Can you work these out from the model? Positions are in its coordinate system, mm. Round coordinates to 2 decimals unless told otherwise and drop trailing zeros. Use a Markdown table: item, result. Add a question column.
```python
from build123d import *

# Parameters (mm, degrees)
SKETCH_1_R      = 2.1
SKETCH_1_R_2    = 3.4
EXTRUDE_1_DEPTH = 1940


with BuildPart() as part:
    # 草图1 → 拉伸1 (new body)
    with BuildSketch(Plane(origin=(0, 0, 0), x_dir=(1, 0, 0), z_dir=(0, 1, 0))):
        with BuildLine():
            Line((6.75, -28), (11, -28))
            Line((11, -28), (11, -30))
            Line((11, -30), (2, -30))
            ThreePointArc((2, -30), (0.585786438, -29.414213562), (0, -28))
            Line((0, -28), (0, -19))
            Line((0, -19), (2, -19))
            Line((2, -19), (2, -23.25))
            Line((2, -23.25), (5.335785999, -23.25))
            Line((5.335785999, -23.25), (9, -19.585785999))
            Line((9, -19.585785999), (9, -10.414214001))
            Line((9, -10.414214001), (5.335785999, -6.75))
            Line((5.335785999, -6.75), (2, -6.75))
            Line((2, -6.75), (2, -11))
            Line((2, -11), (0, -11))
            Line((0, -11), (0, -2))
            ThreePointArc((0, -2), (0.585786438, -0.585786438), (2, 0))
            Line((2, 0), (11, 0))
            Line((11, 0), (11, -2))
            Line((11, -2), (6.75, -2))
            Line((6.75, -2), (6.75, -5.335785999))
            Line((6.75, -5.335785999), (10.414214001, -9))
            Line((10.414214001, -9), (19.585785999, -9))
            Line((19.585785999, -9), (23.25, -5.335785999))
            Line((23.25, -5.335785999), (23.25, -2))
            Line((23.25, -2), (19, -2))
            Line((19, -2), (19, 0))
            Line((19, 0), (28, 0))
            ThreePointArc((28, 0), (29.414213562, -0.585786438), (30, -2))
            Line((30, -2), (30, -11))
            Line((30, -11), (28, -11))
            Line((28, -11), (28, -6.75))
            Line((28, -6.75), (24.664214001, -6.75))
            Line((24.664214001, -6.75), (21, -10.414214001))
            Line((21, -10.414214001), (21, -19.585785999))
            Line((21, -19.585785999), (24.664214001, -23.25))
            Line((24.664214001, -23.25), (28, -23.25))
            Line((28, -23.25), (28, -19))
            Line((28, -19), (30, -19))
            Line((30, -19), (30, -28))
            ThreePointArc((30, -28), (29.414213562, -29.414213562), (28, -30))
            Line((28, -30), (19, -30))
            Line((19, -30), (19, -28))
            Line((19, -28), (23.25, -28))
            Line((23.25, -28), (23.25, -24.664214001))
            Line((23.25, -24.664214001), (19.585785999, -21))
            Line((19.585785999, -21), (10.414214001, -21))
            Line((10.414214001, -21), (6.75, -24.664214001))
            Line((6.75, -24.664214001), (6.75, -28))
        make_face()
        with Locations(Location((3.375, -26.625, 0), (0, 0, 270))):
            Circle(SKETCH_1_R, mode=Mode.SUBTRACT)
        with Locations(Location((26.625, -26.625, 0), (0, 0, 270))):
            Circle(SKETCH_1_R, mode=Mode.SUBTRACT)
        with Locations(Location((15, -15, 0), (0, 0, 270))):
            Circle(SKETCH_1_R_2, mode=Mode.SUBTRACT)
        with Locations(Location((3.375, -3.375, 0), (0, 0, 270))):
            Circle(SKETCH_1_R, mode=Mode.SUBTRACT)
        with Locations(Location((26.625, -3.375, 0), (0, 0, 270))):
            Circle(SKETCH_1_R, mode=Mode.SUBTRACT)
    extrude(amount=EXTRUDE_1_DEPTH)


solid = part.part
```
(1) Suppose I cut it at A-A on y = 1342. Count the separate pieces of the cut face and the enclosed holes in it, and give its area (3 significant figures).
(2) I'm going to push flat-ended pins straight in: pin 1 (1 mm diameter, centred on x = 1, y = 498.5, fed in from +Z); pin 2 (1.6 mm diameter, centred on y = 528.5, z = 29, fed in from +X); pin 3 (5.5 mm diameter, centred on x = 15, z = 15, fed in from +Y); pin 4 (7.5 mm diameter, centred on x = 15, y = 671, fed in from +Z). Where does each tip first touch, or does it pass through?
(3) If I drill on probe 1 along X at (y, z) = (1275, 25.25); probe 2 along Z at (x, y) = (7.25, 810); probe 3 along Z at (x, y) = (3.5, 1173.5), over which ranges is the centre line in solid material (lowest first)? Write a range as [from, to].
Results below:
| question | item | result |
|---|---|---|
| 1 | separate pieces | 1 |
| 1 | enclosed holes | 5 |
| 1 | area | 333 mm² |
| 2 | pin 1 | stops at z = 29.94 |
| 2 | pin 2 | stops at x = 29.99 |
| 2 | pin 3 | passes through |
| 2 | pin 4 | stops at z = 21 |
| 3 | probe 1 | x = [0, 1.79], [4.96, 6.75], [23.25, 25.04], [28.21, 30] |
| 3 | probe 2 | z = [0, 2], [5.84, 8.66], [21.34, 24.16], [28, 30] |
| 3 | probe 3 | z = [0, 1.28], [5.47, 6.75], [23.25, 24.53], [28.72, 30] |
